Check sheet for the modelled part. Datum: model origin and axes. Units: mm. A direction names the side the tool comes from. Coordinates: 2 decimals unless noted, no trailing zeros. Write each loop counter-clockwise with the first axis right and the second up, starting at its lowest first coordinate (ties: lowest second). Pieces come first, ordered by that corner, then holes. Notation, with made-up numbers: (57, -17.75) -> (83, -17.75) arc R29 cw to (83, 17.25) -> close; hole circle Ø6 at (5.25, 35.25). An arc over 180 degrees is marked (long way). One line per item, written item: value. Start each with the question number.
1) Set-up check for faces 5 (the flat face through (6, -1311, -112.5)), 6 (the flat face through (438, 907, -90)), 7 (the flat face through (-376, 957, -100)), 8 (the cylindrical face through (388.742, 1381.266, -234.964)), 9 (the flat face through (5, -651, -100)): record each of +Z, -Z, +X, -X, +Y, -Y from which the full face is reachable in a straight line by a thin tool's end or side.
2) Sectioned sample at D-D on y = 11.5. Enter the section's corners in (x, z).
3) Draft check along X on faces 1 (the flat face through (376, 20, 92.5)), 2 (the flat face through (-377, 20, -92.5)), 3 (the flat face through (362.5, 1276, -164)), 4 (the flat face through (-407, -1400, 0)). Enter one of: +X half, -X half, draft (parallel to the pull), parting line (faces both ways), or undercut.
4) Gauge pin test, flat ends, axial feed: P1, Ø4, axis at x = -382, y = -1395.5, coming from the -Z side; P2, Ø10, axis at x = -48.5, z = -106.5, coming from the -Y side; P3, Ø3, axis at y = -847, z = -95.5, coming from the +X side. Record the tip position at first contact, or that the pin passes through.
5) Sectioned sample at C-C on x = 92.5. Enter the section's corners in (y, z), plus the area to 3 significant figures.
6) Sectioned sample at B-B on z = -2.5. Enter the section's corners in (x, y).
7) Scan lines: line 1 along X through (y, z) = (1183.75, -182); line 2 along Z through (x, y) = (384, 1180); line 3 along X through (y, z) = (-1262, -89.5). Record each from-to range of solid material in increasing order. Write a range as [from, to].
```python
from build123d import *

# Parameters (mm, degrees)
SIDE_CHANNEL_RAIL_L2800_DEPTH = 1400
TOP_CAP_SKETCH_W              = 50
TOP_CAP_SKETCH_H              = 12.5
TOP_CAP_PLATE_DEPTH           = 1000
SIDE_BRACKET_DEPTH            = 38
CROSS_BAR_SKETCH_W            = 806
CROSS_BAR_SKETCH_H            = 150
CROSS_BAR_DEPTH               = 12.5
CROSS_BAR_PATTERN_660_COUNT   = 2
CROSS_BAR_PATTERN_660_PITCH   = 660
CROSS_BAR_PATTERN_1970_COUNT  = 2
CROSS_BAR_PATTERN_1970_PITCH  = 1970
HANGER_PLATE_SKETCH_W         = 12.5
HANGER_PLATE_SKETCH_H         = 127
HANGER_PLATE_DEPTH            = 175
HANGER_TAB_SKETCH_W           = 53
HANGER_TAB_SKETCH_H           = 127
HANGER_TAB_SKETCH_R           = 8.75
HANGER_TAB_DEPTH              = 12.5
HANGER_TAB_FILLET_R12_5_R     = 12.5


with BuildPart() as part:
    # Side Channel Profile Sketch → Side Channel Rail L2800 (new, symmetric)
    with BuildSketch(Plane(origin=(0, 0, 0), x_dir=(1, 0, 0), z_dir=(0, 1, 0))):
        with BuildLine():
            Line((350, 100), (403, 100))
            ThreePointArc((403, 100), (410.071067812, 97.071067812), (413, 90))
            Line((413, 90), (413, -90))
            ThreePointArc((413, -90), (410.071067812, -97.071067812), (403, -100))
            Line((403, -100), (350, -100))
            Line((350, -100), (350, -92.5))
            Line((350, -92.5), (403, -92.5))
            ThreePointArc((403, -92.5), (404.767766953, -91.767766953), (405.5, -90))
            Line((405.5, -90), (405.5, 90))
            ThreePointArc((405.5, 90), (404.767766953, 91.767766953), (403, 92.5))
            Line((403, 92.5), (350, 92.5))
            Line((350, 92.5), (350, 100))
        make_face()
    extrude(amount=SIDE_CHANNEL_RAIL_L2800_DEPTH, both=True)

    # Top Cap Sketch → Top Cap Plate (add)
    with BuildSketch(Plane(origin=(0, 1400, 0), x_dir=(1, 0, 0), z_dir=(0, 1, 0))):
        with Locations((438, 83.75)):
            Rectangle(TOP_CAP_SKETCH_W, TOP_CAP_SKETCH_H)
    extrude(amount=-TOP_CAP_PLATE_DEPTH)


with BuildPart() as body_2:
    # Side Rail Mirror: mirrored copy
    add(part.part.mirror(Plane(origin=(0, 0, 0), x_dir=(0, 0, 1), z_dir=(1, 0, 0))))


with BuildPart() as part_1:
    add(part.part)

    add(body_2.part)  # Side Bracket merges body 2
    # Bracket Sketch → Side Bracket (add)
    with BuildSketch(Plane(origin=(0, 1400, 0), x_dir=(1, 0, 0), z_dir=(0, 1, 0))):
        with BuildLine():
            Line((-403, 100), (403, 100))
            Line((403, 100), (403, 200))
            ThreePointArc((403, 200), (388.355339059, 235.355339059), (353, 250))
            Line((353, 250), (-353, 250))
            ThreePointArc((-353, 250), (-388.355339059, 235.355339059), (-403, 200))
            Line((-403, 200), (-403, 100))
        make_face()
    extrude(amount=-SIDE_BRACKET_DEPTH)

    # Cross Bar Sketch → Cross Bar (add)
    with BuildSketch(Plane(origin=(0, 0, -100), x_dir=(-1, 0, 0), z_dir=(0, 0, -1))):
        with Locations((0, -1312.5)):
            Rectangle(CROSS_BAR_SKETCH_W, CROSS_BAR_SKETCH_H)
    cross_bar = extrude(amount=CROSS_BAR_DEPTH)

    # Cross Bar Pattern 660: Cross Bar ×2
    with Locations(*[(0, i * CROSS_BAR_PATTERN_660_PITCH, 0) for i in range(1, CROSS_BAR_PATTERN_660_COUNT)]):
        add(cross_bar)

    # Cross Bar Pattern 1970: Cross Bar ×2
    with Locations(*[(0, i * CROSS_BAR_PATTERN_1970_PITCH, 0) for i in range(1, CROSS_BAR_PATTERN_1970_COUNT)]):
        add(cross_bar)

    # Hanger Plate Sketch → Hanger Plate (add)
    with BuildSketch(Plane.XZ.offset(-1362)):
        with Locations((-356.25, -163.5)):
            Rectangle(HANGER_PLATE_SKETCH_W, HANGER_PLATE_SKETCH_H)
    extrude(amount=HANGER_PLATE_DEPTH)

    # Hanger Tab Sketch → Hanger Tab (add)
    with BuildSketch(Plane.XZ.offset(-1187)):
        with Locations((-376.5, -163.5)):
            Rectangle(HANGER_TAB_SKETCH_W, HANGER_TAB_SKETCH_H)
        with Locations(Location((-384, -182, 0), (0, 0, 270))):
            Circle(HANGER_TAB_SKETCH_R, mode=Mode.SUBTRACT)
    extrude(amount=HANGER_TAB_DEPTH)

    # Hanger Tab Fillet R12.5
    hanger_tab_fillet_r12_5_edges = [part_1.edges().sort_by_distance(p)[0] for p in [
        (-403, 1180.75, -227),
    ]]
    fillet(hanger_tab_fillet_r12_5_edges, radius=HANGER_TAB_FILLET_R12_5_R)

    # Side Bracket Mirror: part across plane


with BuildPart() as part_2:
    add(part_1.part)
    add(part_1.part.mirror(Plane(origin=(0, 0, 0), x_dir=(0, 0, 1), z_dir=(1, 0, 0))))


solid = part_2.part
```
Answers:
1. face 5: -Z, +X, -X, -Y
1. face 6: -Z, +X, +Y, -Y
1. face 7: -Z, +X, -X
1. face 8: -Z, +X, +Y
1. face 9: +Z, +Y, -Y
2. outline: (-413, -90) arc R10 ccw to (-403, -100) -> (-350, -100) -> (-350, -92.5) -> (-403, -92.5) arc R2.5 cw to (-405.5, -90) -> (-405.5, 90) arc R2.5 cw to (-403, 92.5) -> (-350, 92.5) -> (-350, 100) -> (-403, 100) arc R10 ccw to (-413, 90) -> close; (350, -100) -> (403, -100) arc R10 ccw to (413, -90) -> (413, 90) arc R10 ccw to (403, 100) -> (350, 100) -> (350, 92.5) -> (403, 92.5) arc R2.5 cw to (405.5, 90) -> (405.5, -90) arc R2.5 cw to (403, -92.5) -> (350, -92.5) -> close
3. face 1: undercut
3. face 2: undercut
3. face 3: +X half
3. face 4: draft
4. P1: stops at z = -100
4. P2: stops at y = -1387.5
4. P3: stops at x = 412.17
5. outline: (-1387.5, -112.5) -> (-1237.5, -112.5) -> (-1237.5, -100) -> (-1387.5, -100) -> close; (-727.5, -112.5) -> (-577.5, -112.5) -> (-577.5, -100) -> (-727.5, -100) -> close; (582.5, -112.5) -> (732.5, -112.5) -> (732.5, -100) -> (582.5, -100) -> close; (1362, -250) -> (1400, -250) -> (1400, -100) -> (1362, -100) -> close
5. area: 11,300 mm2
6. outline: (-413, -1400) -> (-405.5, -1400) -> (-405.5, 1400) -> (-413, 1400) -> close; (405.5, -1400) -> (413, -1400) -> (413, 1400) -> (405.5, 1400) -> close
7. line 1: x = [-403, -392.75], [-375.25, -350], [350, 375.25], [392.75, 403]
7. line 2: z = [-227, -190.75], [-173.25, -92.5], [92.5, 100]
7. line 3: x = [-413, -405.5], [405.5, 413]
